Model file for the job. Use its own axes, mm. Face numbers are marked on the shaded views. A direction names the side the tool comes from. Round coordinates to 2 decimals unless told otherwise and drop trailing zeros. Order: outer loops, then holes, each group sorted by start corner. A loop starts at its lowest first (then second) coordinate and runs counter-clockwise, first axis right, second up. Notation, with made-up numbers: (-39.5, -15) - (-9.5, -15) arc R28 cw to (-9.5, 10) - close; hole circle Ø10 at (33, 56.25). An arc over 180 degrees is marked (long way). Put each result on its own line as item: value. Start each with the question number.
Item 1: Saw through at D-D on x = 0. List the corners of the cut face in (y, z).
Item 2: Probe probe 1 along Y at (x, z) = (85, 45.5); probe 2 along X at (y, z) = (232, 67.5); probe 3 along Y at (x, z) = (31, 44). List the from-to ranges inside material, lowest first.
Item 3: Saw through at C-C on z = 0. List the corners of the cut face in (x, y), plus the area to 3 significant figures.
Item 4: Pin check, flat tips, straight feed: pin 1 Ø1.5 at (x, y) = (-55, 228) entering from -Z; pin 2 Ø1 at (y, z) = (67, 25.5) entering from +X; pin 3 Ø2.5 at (x, z) = (51.5, 8.5) entering from +Y. Stop position of each tip, or through.
Item 5: Mould opens along X. For the marked faces 5, 6 and 7 say: pulls with the +X half, pulls with the -X half, needs draft (parallel to the pull), parting line crosses it, or undercut.
Item 6: Saw through at A-A on z = -73. List the corners of the cut face in (x, y), plus the area to 3 significant figures.
Item 7: Which spindle directions (+Z, -Z, +X, -X, +Y, -Y) get a long thin tool onto all of the face, cutting with end or side? Do the marked faces 1, 2, 3 and 4. Say none if no direction does.
Item 8: Saw through at B-B on x = -49. List the corners of the cut face in (y, z), plus the area to 3 significant figures.
```python
from build123d import *

# Parameters (mm, degrees)
SKETCH1_R                  = 45
BOSS_EXTRUDE1_DEPTH        = 180
BOSS_EXTRUDE2_DEPTH        = 90
BOSS_EXTRUDE2_DEPTH_BACK   = 90
SKETCH3_R                  = 10
BOSS_EXTRUDE2_2_DEPTH      = 90
BOSS_EXTRUDE2_2_DEPTH_BACK = 90
BOSS_EXTRUDE3_DEPTH        = 30
BOSS_EXTRUDE3_DEPTH_BACK   = 30
SKETCH5_R                  = 54.083269132
BOSS_EXTRUDE4_DEPTH        = 10
SKETCH6_R                  = 15
BOSS_EXTRUDE5_DEPTH        = 3
BOSS_EXTRUDE6_START        = 3
SKETCH7_R                  = 15
BOSS_EXTRUDE6_DEPTH        = 3


with BuildPart() as part:
    # Sketch1 → Boss-Extrude1 (new body)
    with BuildSketch(Plane(origin=(0, 0, 0), x_dir=(1, 0, 0), z_dir=(0, 1, 0))):
        with Locations(Location((0, 0, 0), (0, 0, 90))):
            Circle(SKETCH1_R)
    extrude(amount=BOSS_EXTRUDE1_DEPTH)



with BuildPart() as body_2:
    # Sketch3 → Boss-Extrude2 (new, two sides: drawn at the far end of the back side and taken through both)
    with BuildSketch(Plane.XY.offset(-BOSS_EXTRUDE2_DEPTH_BACK)):
        with Locations((85, 230)):
            Circle(SKETCH3_R)
    extrude(amount=BOSS_EXTRUDE2_DEPTH + BOSS_EXTRUDE2_DEPTH_BACK)


with BuildPart() as body_3:
    # Sketch3 → Boss-Extrude2 2 (new, two sides: drawn at the far end of the back side and taken through both)
    with BuildSketch(Plane.XY.offset(-BOSS_EXTRUDE2_2_DEPTH_BACK)):
        with Locations((-85, 230)):
            Circle(SKETCH3_R)
    extrude(amount=BOSS_EXTRUDE2_2_DEPTH + BOSS_EXTRUDE2_2_DEPTH_BACK)


with BuildPart() as part_1:
    add(part.part)

    add(body_2.part)  # Boss-Extrude3 merges body 2

    add(body_3.part)  # Boss-Extrude3 merges body 3
    # Sketch4 → Boss-Extrude3 (add, two sides: drawn at the far end of the back side and taken through both)
    with BuildSketch(Plane.XY.offset(-BOSS_EXTRUDE3_DEPTH_BACK)):
        with BuildLine():
            Line((-45, 180), (-10, 180))
            ThreePointArc((-10, 180), (-43.69905694, 199.308584519), (-67.5, 230))
            ThreePointArc((-67.5, 230), (-98.082305532, 241.623393737), (-82.940375083, 212.621624207))
            ThreePointArc((-82.940375083, 212.621624207), (-66.424952125, 193.455813577), (-45, 180))
        make_face()
        with BuildLine():
            Line((10, 180), (45, 180))
            ThreePointArc((45, 180), (60.253550288, 202.66599047), (67.528581994, 229.00022359))
            ThreePointArc((67.528581994, 229.00022359), (102.492853042, 230.500092441), (67.5, 230))
            ThreePointArc((67.5, 230), (43.69905694, 199.308584519), (10, 180))
        make_face()
    extrude(amount=BOSS_EXTRUDE3_DEPTH + BOSS_EXTRUDE3_DEPTH_BACK)

    # Sketch5 → Boss-Extrude4 (add)
    with BuildSketch(Plane.XZ.offset(-180)):
        with Locations(Location((0, 0, 0), (0, 0, 33.690067526))):
            Circle(SKETCH5_R)
    extrude(amount=BOSS_EXTRUDE4_DEPTH)

    # Sketch6 → Boss-Extrude5 (add)
    with BuildSketch(Plane.XY.offset(30)):
        with Locations((-85, 230)):
            Circle(SKETCH6_R)
        with Locations(Location((85, 230, 0), (0, 0, 180))):
            Circle(SKETCH6_R)
    extrude(amount=BOSS_EXTRUDE5_DEPTH)

    # Sketch7 → Boss-Extrude6 (add)
    with BuildSketch(Plane(origin=(0, 0, -30), x_dir=(-1, 0, 0), z_dir=(0, 0, -1)).offset(BOSS_EXTRUDE6_START)):
        with Locations((-85, 230)):
            Circle(SKETCH7_R)
        with Locations(Location((85, 230, 0), (0, 0, 180))):
            Circle(SKETCH7_R)
    extrude(amount=-BOSS_EXTRUDE6_DEPTH)

    # Sketch8 → Revolve1 (revolve)
    with BuildSketch(Plane(origin=(-85, 0, 0), x_dir=(0, 0, -1), z_dir=(1, 0, 0)), mode=Mode.PRIVATE) as revolve1_sk:
        Polygon((-33, 240.5), (-33, 258.5), (-36, 260.5), (-85, 260.5), (-88, 258.5), (-88, 240.5), align=None)
    revolve1 = revolve(revolve1_sk.sketch.rotate(Axis((-85, 230, 33), (0, 0, 1)), 90), axis=Axis((-85, 230, 33), (0, 0, 1)))

    # Mirror1: Revolve1 across plane
    add(revolve1.mirror(Plane(origin=(0, 0, 0), x_dir=(0, 0, 1), z_dir=(1, 0, 0))))

    # Mirror2: Revolve1 across plane
    add(revolve1.mirror(Plane.XY))

    # Mirror2 copy 1 sketch → Mirror2 copy 1 (revolve)
    with BuildSketch(Plane.ZY.offset(-85)):
        Polygon((-33, 240.5), (-33, 258.5), (-36, 260.5), (-85, 260.5), (-88, 258.5), (-88, 240.5), align=None)
    revolve(axis=Axis((85, 230, -33), (0, 0, -1)))


solid = part_1.part
```
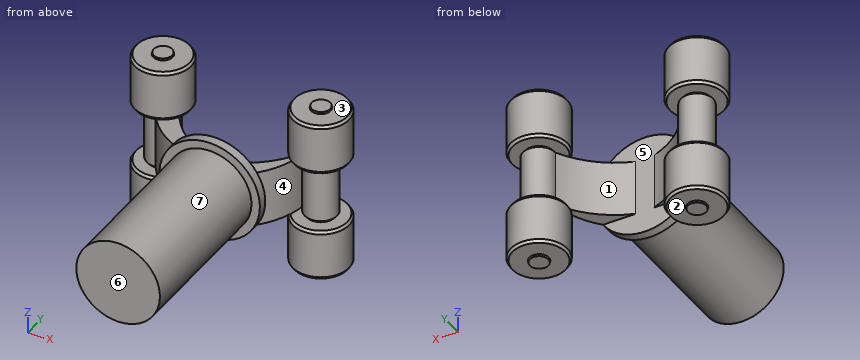
Results found:
1. outline: (0, -45) - (170, -45) - (170, -54.08) - (180, -54.08) - (180, 54.08) - (170, 54.08) - (170, 45) - (0, 45) - close
2. probe 1: y = 199.5 to 219.5, 220 to 240, 240.5 to 260.5
2. probe 2: x = -115.43 to -95.31, -94.8 to -75.2, -74.69 to -54.57, 54.57 to 74.69, 75.2 to 94.8, 95.31 to 115.43
2. probe 3: y = 170 to 180
3. outline: (-82.94, 212.62) arc R85 ccw to (-45, 180) - (-54.08, 180) - (-54.08, 170) - (-45, 170) - (-45, 0) - (45, 0) - (45, 170) - (54.08, 170) - (54.08, 180) - (45, 180) arc R85 ccw to (67.53, 229) arc R17.5 ccw (long way) to (67.5, 230) arc R100 cw to (10, 180) - (-10, 180) arc R100 cw to (-67.5, 230) arc R17.5 ccw (long way) to start
3. area: 20,100 mm²
4. pin 1: stops at z = -86.78
4. pin 2: stops at x = 37.42
4. pin 3: stops at y = 208.25
5. face 5: undercut
5. face 6: needs draft
5. face 7: parting line crosses it
6. outline: circle Ø61 at (-85, 230); circle Ø20 at (-85, 230); circle Ø61 at (85, 230); circle Ø20 at (85, 230); hole circle Ø21 at (-85, 230); hole circle Ø21 at (85, 230)
6. area: 5,780 mm²
7. face 1: +Y
7. face 2: -Z
7. face 3: +Z
7. face 4: none
8. outline: (170, -22.89) - (180, -22.89) - (180, 22.89) - (170, 22.89) - close; (181.87, -30) - (204.27, -30) - (204.27, 30) - (181.87, 30) - close
8. area: 1,800 mm²
